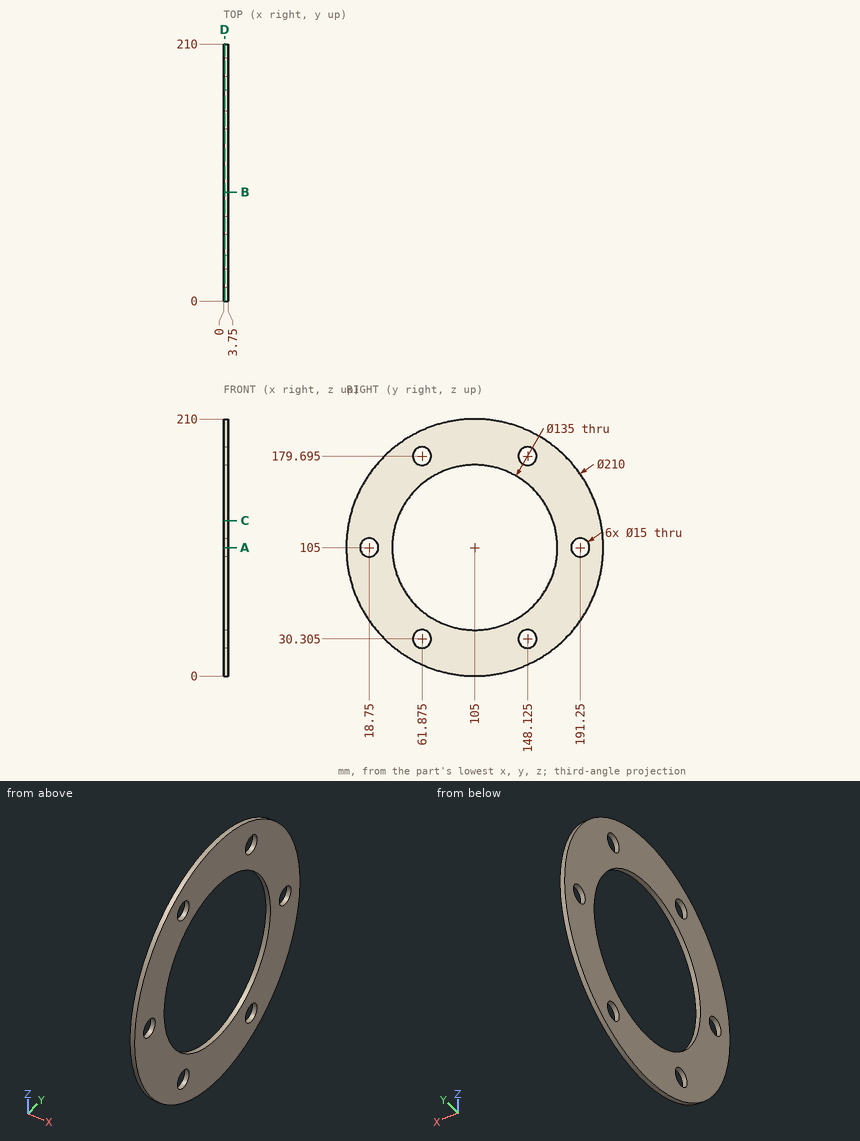
The figure shows three views and two pictorial views of one solid part (mm, origin at its lowest corner). Answer the questions. Give positions to 0.01 mm unless a question says otherwise; leave off trailing zeros. Order: outer loops, then holes, each group sorted by start corner. A loop starts at its lowest first (then second) coordinate and runs counter-clockwise, first axis right, second up. Notation, with made-up numbers: (-16.75, 42.25) -> (38.25, 42.25) arc R16 cw to (38.25, 71.25) -> close; hole circle Ø10 at (-34, -23). An arc over 180 degrees is marked (long way). One line per item, written item: value.
1) Flat-ended cylindrical pins translate along their axes: P1, Ø1, axis at x = 1, y = 91, coming from the +Z side; P2, Ø9, axis at y = 148.12, z = 30.31, coming from the +X side. Find the tip coordinate at first contact, or state that the pin passes through.
Reported:
P1: stops at z = 209.13
P2: passes through
2) Find section C-C, the plane z = 127. Determine the outline of the cut face in (x, y).
Reported:
outline: (0, 2.33) -> (3.75, 2.33) -> (3.75, 41.19) -> (0, 41.19) -> close; (0, 168.81) -> (3.75, 168.81) -> (3.75, 207.67) -> (0, 207.67) -> close
3) Find section B-B, the plane y = 89. Determine the outline of the cut face in (x, z).
Reported:
outline: (0, 1.23) -> (3.75, 1.23) -> (3.75, 39.42) -> (0, 39.42) -> close; (0, 170.58) -> (3.75, 170.58) -> (3.75, 208.77) -> (0, 208.77) -> close
4) Find section A-A, the plane z = 105. Determine the outline of the cut face in (x, y), plus the area to 3 significant figures.
Reported:
outline: (0, 0) -> (3.75, 0) -> (3.75, 11.25) -> (0, 11.25) -> close; (0, 26.25) -> (3.75, 26.25) -> (3.75, 37.5) -> (0, 37.5) -> close; (0, 172.5) -> (3.75, 172.5) -> (3.75, 183.75) -> (0, 183.75) -> close; (0, 198.75) -> (3.75, 198.75) -> (3.75, 210) -> (0, 210) -> close
area: 169 mm^2
5) Find the intervals of material crossed by line 1 (Z direction, x = 2.15, y = 57.5) (1 decimal); line 2 (Y direction, x = 0.65, z = 30) (1 decimal); line 3 (Y direction, x = 1, z = 146) (1 decimal), in increasing order.
Reported:
line 1: z = 11.4 to 24.2, 36.4 to 57, 153 to 173.6, 185.8 to 198.6
line 2: y = 31.5 to 54.4, 69.4 to 140.6, 155.6 to 178.5
line 3: y = 8.3 to 51.4, 158.6 to 201.7
6) Find section D-D, the plane x = 0.8. Count the separate pieces of the cut face and the enclosed holes in it, plus the area to 3 significant figures.
Reported:
separate pieces: 1
enclosed holes: 7
area: 19,300 mm^2
